The drawing under review shows one solid part. Ordinate dimensions are in mm from its lowest x, y, z. A direction names the side the tool comes from. Coordinates: 2 decimals unless noted, no trailing zeros. Loops run counter-clockwise (first coordinate to the right, second up) from the corner with the lowest first, then second, coordinate; pieces in that order, holes last. Notation, with made-up numbers: M -13.75,-20.5 L 33.25,-20.5 A18 ccw 33.25,-11.5 Z; hole C 5,-14.75 d9. An arc over 180 degrees is marked long. Return JSON: item names as keys, results as strings.
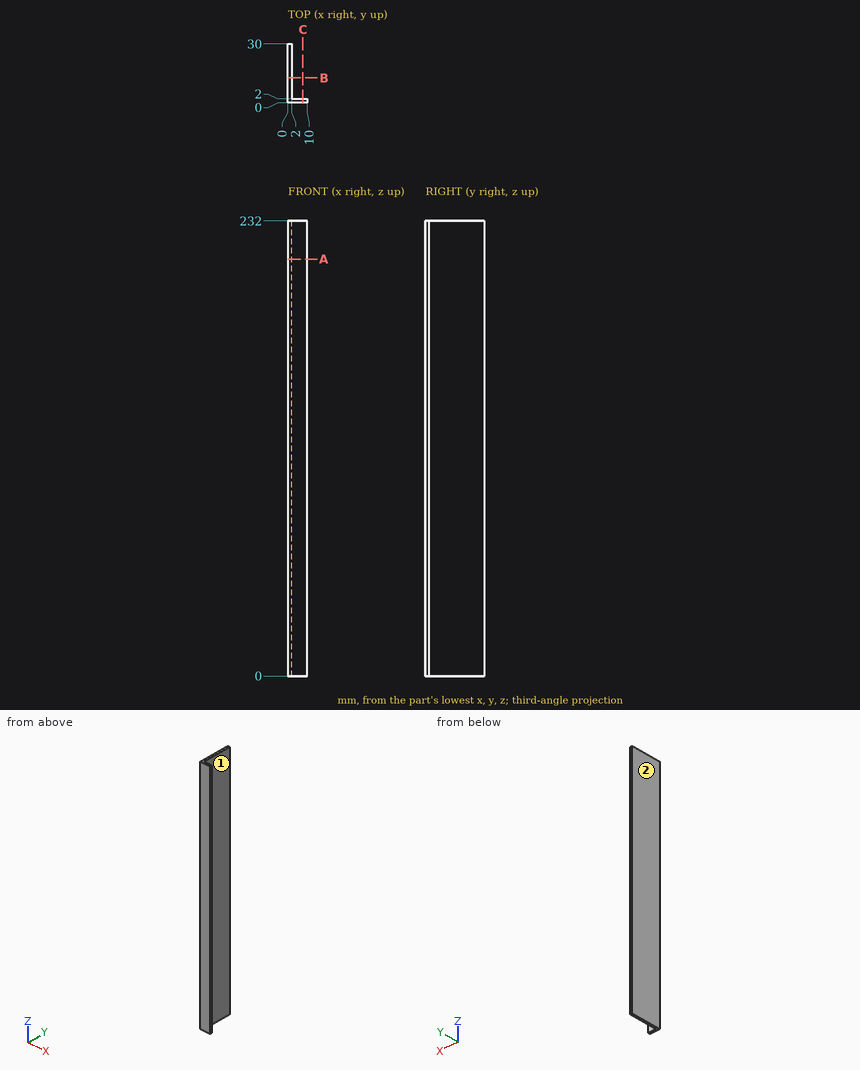
1. Add section A-A on z = 212.5. Give the boundary of the cut face in (x, y).
Check values:
{"outline": "M 0,0 L 10,0 L 10,2 L 2,2 L 2,30 L 0,30 Z"}
2. Add section B-B on y = 12.75. Give the boundary of the cut face in (x, z), plus the area to 3 significant figures.
Check values:
{"outline": "M 0,0 L 2,0 L 2,232 L 0,232 Z", "area": "464 mm²"}
3. To check wall thickness, follow line 1 (Y direction, x = 9, z = 208). State the ranges of the line that lie inside material, in increasing order.
Check values:
{"line 1": "0 to 2"}
4. Machinability: for the marked faces 1 and 2, which of the approach directions +Z, -Z, +X, -X, +Y, -Y give a long, thin tool a straight path to every point of the face, cutting with its end or side? Answer none if there is none.
Check values:
{"face 1": "+Z, -Z, +X, +Y", "face 2": "+Z, -Z, -X, +Y, -Y"}
5. Insertion check: pin 1 Ø8 at (y, z) = (19, 81.5) entering from -X; pin 2 Ø3 at (y, z) = (4, 151) entering from +X. Each pin has a flat end and moves straight along its axis. Give the tip position at first contact, or say it passes through.
Check values:
{"pin 1": "x = 0", "pin 2": "x = 2"}
